from build123d import *

# Parameters (mm, degrees)
SKETCH1_R          = 1
BASE_EXTRUDE_DEPTH = 1.2


with BuildPart() as part:
    # Sketch1 → Base-Extrude (new body)
    with BuildSketch(Plane.XY):
        with BuildLine():
            Line((-4.17437466, -10.077831919), (-5.147092165, -12.426179712))
            ThreePointArc((-5.147092165, -12.426179712), (0, 13.45), (5.147092165, -12.426179712))
            Line((5.147092165, -12.426179712), (4.17437466, -10.077831919))
            ThreePointArc((4.17437466, -10.077831919), (4.821639244, -7.712836035), (7.273294145, -7.752145343))
            ThreePointArc((7.273294145, -7.752145343), (8.165152835, -8.007621744), (8.972639508, -7.550844571))
            ThreePointArc((8.972639508, -7.550844571), (0, 10.75), (-8.972639508, -7.550844571))
            ThreePointArc((-8.972639508, -7.550844571), (-8.165152835, -8.007621744), (-7.273294145, -7.752145343))
            ThreePointArc((-7.273294145, -7.752145343), (-4.821639244, -7.712836035), (-4.17437466, -10.077831919))
        make_face()
        with Locations((-5.909254613, -9.03995077)):
            Circle(SKETCH1_R, mode=Mode.SUBTRACT)
        with Locations(Location((5.909254613, -9.03995077, 0), (0, 0, 180))):
            Circle(SKETCH1_R, mode=Mode.SUBTRACT)
    extrude(amount=BASE_EXTRUDE_DEPTH)


solid = part.part
Input: part model. Units: mm. Frame: model coordinates. A direction names the side the tool comes from. Coordinates: 2 decimals unless noted, no trailing zeros. Loops run counter-clockwise (first coordinate to the right, second up) from the corner with the lowest first, then second, coordinate; pieces in that order, holes last. Notation, with made-up numbers: (-7.75, 3.25) - (44.25, 3.25) arc R14 cw to (44.25, 28.25) - close; hole circle Ø5 at (-29, -3.5). An arc over 180 degrees is marked (long way). Answer in a Markdown table with one row per item. Add a question column.
Item 1: Line query: line 1 along X through (y, z) = (-6.75, 0.4); line 2 along X through (y, z) = (-2, 0.75); line 3 along Y through (x, z) = (7, 0.3). Output: solid intervals per line, ascending. Write a range as [from, to].
Item 2: Mould query, pull axis X, two halves, no side actions, for faces 4 (the flat face through (0, 11, 0)), 5 (the cylindrical face through (5.45, -8.15, 0.59)), 6 (the cylindrical face through (-0.52, 13.44, 0.59)). Classes: released by +X, released by -X, zero draft, split by the parting line, or undercut.
Item 3: Section query D-D on x = 0. Return the cut outline in (y, z), then the cut area to 3 significant figures.
Item 4: Access query for faces 1 (the cylindrical face through (-8.178, -8.006, 0.592)), 2 (the flat face through (0, 11, 1.2)), 3 (the flat face through (4.67, -11.27, 0.59)). Directions: +Z, -Z, +X, -X, +Y, -Y. A direction counts if a zero-diameter tool reaches every point of the face in a straight line with its end or side. Return the directions, or none.
Item 5: Section query A-A on y = 2.25. Return the cut outline in (x, z).
Item 6: Section query C-C on z = 0.7. Return the cut outline in (x, y).
Item 7: Section query B-B on x = 8.25. Return the cut outline in (y, z), then the cut area to 3 significant figures.
Item 8: Contact query for a flat-ended pin moving along its axis: P1, Ø1, axis at x = -6.5, y = -5.5, coming from the -Z side. Output: stop coordinate, or through.
Recorded:
| question | item | result |
|---|---|---|
| 1 | line 1 | [-11.63, -9.54], [9.54, 11.63] |
| 1 | line 2 | [-13.3, -11.26], [11.26, 13.3] |
| 1 | line 3 | [-11.48, -7.57], [8.33, 11.48] |
| 2 | face 4 | zero draft |
| 2 | face 5 | undercut |
| 2 | face 6 | split by the parting line |
| 3 | outline | (10.75, 0) - (13.45, 0) - (13.45, 1.2) - (10.75, 1.2) - close |
| 3 | area | 3.24 mm^2 |
| 4 | face 1 | +Z, -Z |
| 4 | face 2 | +Z, +X, -X, +Y, -Y |
| 4 | face 3 | +Z, -Z, -Y |
| 5 | outline | (-13.26, 0) - (-10.99, 0) - (-10.99, 1.2) - (-13.26, 1.2) - close; (10.99, 0) - (13.26, 0) - (13.26, 1.2) - (10.99, 1.2) - close |
| 6 | outline | (-8.97, -7.55) arc R11.35 cw (long way) to (8.97, -7.55) arc R1.2 cw to (7.27, -7.75) arc R2 ccw to (4.17, -10.08) - (5.15, -12.43) arc R13.45 ccw (long way) to (-5.15, -12.43) - (-4.17, -10.08) arc R2 ccw to (-7.27, -7.75) arc R1.2 cw to start; hole circle Ø2 at (-5.91, -9.04); hole circle Ø2 at (5.91, -9.04) |
| 7 | outline | (-10.62, 0) - (-7.99, 0) - (-7.99, 1.2) - (-10.62, 1.2) - close; (7.19, 0) - (10.62, 0) - (10.62, 1.2) - (7.19, 1.2) - close |
| 7 | area | 7.27 mm^2 |
| 8 | P1 | through |
